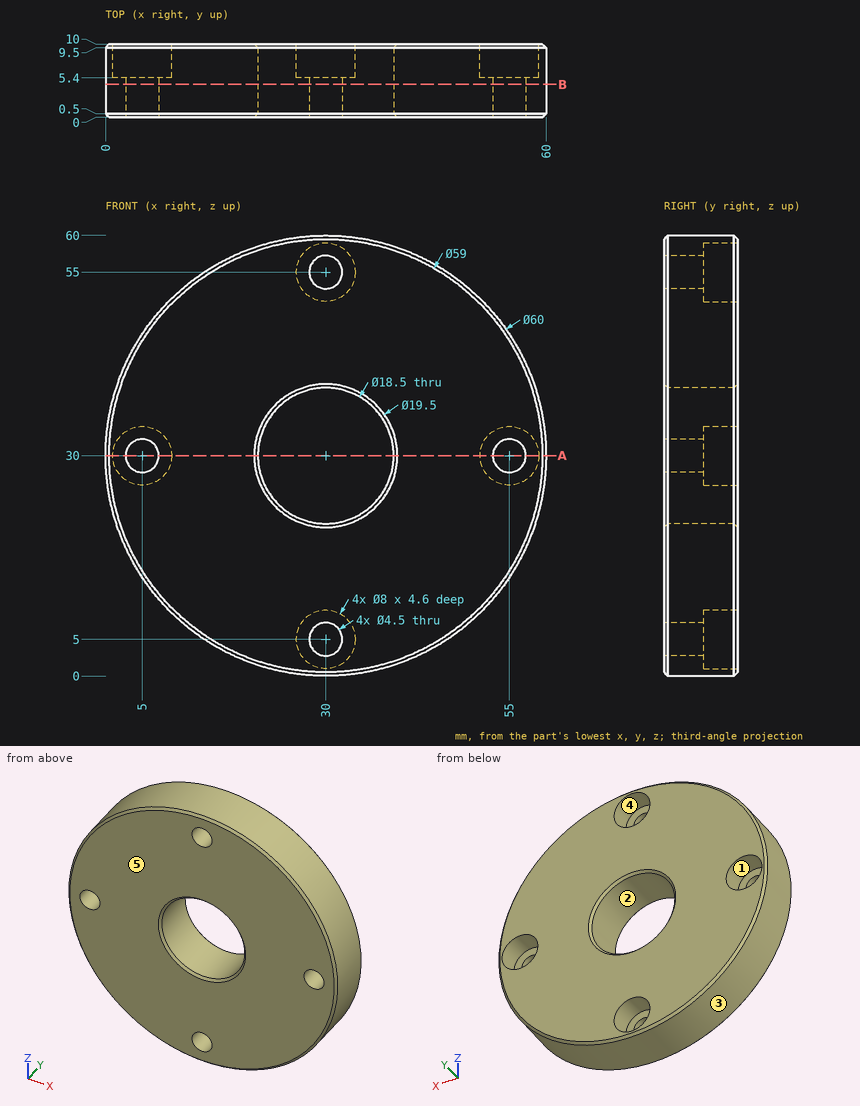
The figure shows three views and two pictorial views of one solid part (mm, origin at its lowest corner). Answer the questions. A direction names the side the tool comes from. Coordinates: 2 decimals unless noted, no trailing zeros. Write each loop counter-clockwise with the first axis right and the second up, starting at its lowest first coordinate (ties: lowest second). Pieces come first, ordered by that corner, then holes. Notation, with made-up numbers: (0.5, 56.25) -> (7.5, 56.25) arc R19 cw to (7.5, 85.25) -> close; hole circle Ø9 at (14.25, 20.25). An arc over 180 degrees is marked (long way). Return JSON: item names as keys, results as strings.
(1) Consider line 1 along X through (y, z) = (4.25, 30); line 2 along X through (y, z) = (7.2, 30); line 3 along Y through (x, z) = (52, 27.5). Determine where each line is inside the solid, lowest interval first. Write a range as from..to.
Answers below:
{"line 1": "0..2.75, 7.25..20.75, 39.25..52.75, 57.25..60", "line 2": "0..1, 9..20.75, 39.25..51, 59..60", "line 3": "0..5.4"}
(2) The part is cut by section B-B on y = 4.5. Give the vertices of the cut face in (x, z).
Answers below:
{"outline": "circle Ø60 at (30, 30); hole circle Ø4.5 at (5, 30); hole circle Ø18.5 at (30, 30); hole circle Ø4.5 at (30, 5); hole circle Ø4.5 at (30, 55); hole circle Ø4.5 at (55, 30)"}
(3) The part is cut by section A-A on z = 30. State how many separate pieces and enclosed holes the cut face has, then the cut area to 3 significant figures.
Answers below:
{"separate pieces": "4", "enclosed holes": "0", "area": "292 mm^2"}
(4) Which of the six approach directions +Z, -Z, +X, -X, +Y, -Y give full straight-line access (tool end or side, diameter ignored) to the marked faces 1 and 2?
Answers below:
{"face 1": "+Y", "face 2": "+Y, -Y"}
(5) Each of these flat-tipped pins is pushed along its axis until it touches: P1, Ø4, axis at y = 4.5, z = 27, coming from the -X side; P2, Ø1, axis at y = 4, z = 31.5, coming from the +X side; P3, Ø1, axis at x = 49, y = 8.5, coming from the +Z side. Where does it stop, or does it pass through?
Answers below:
{"P1": "x = 0.02", "P2": "x = 59.98", "P3": "z = 53.62"}
(6) For a pull along Z with two mould halves and no side action, classify the marked faces 3, 4 and 5 as pulls with the +Z half, pulls with the -Z half, needs draft (parallel to the pull), parting line crosses it, or undercut.
Answers below:
{"face 3": "parting line crosses it", "face 4": "undercut", "face 5": "needs draft"}
